from build123d import *

# Parameters (mm, degrees)
SKETCH_1_R      = 925
SKETCH_1_W      = 122
SKETCH_1_H      = 122
EXTRUDE_1_DEPTH = 12


with BuildPart() as part:
    # 草图1 → 凸台-拉伸1 (new body)
    with BuildSketch(Plane(origin=(0, 0, 0), x_dir=(1, 0, 0), z_dir=(0, 1, 0))):
        with Locations(Location((0, 0, 0), (0, 0, 270))):
            Circle(SKETCH_1_R)
        with BuildLine():
            Line((-648.074069841, 425), (-425, 425))
            Line((-425, 425), (-425, 648.074069841))
            ThreePointArc((-425, 648.074069841), (0, 775), (425, 648.074069841))
            Line((425, 648.074069841), (425, 425))
            Line((425, 425), (648.074069841, 425))
            ThreePointArc((648.074069841, 425), (775, 0), (648.074069841, -425))
            Line((648.074069841, -425), (425, -425))
            Line((425, -425), (425, -648.074069841))
            ThreePointArc((425, -648.074069841), (0, -775), (-425, -648.074069841))
            Line((-425, -648.074069841), (-425, -425))
            Line((-425, -425), (-648.074069841, -425))
            ThreePointArc((-648.074069841, -425), (-775, 0), (-648.074069841, 425))
        make_face(mode=Mode.SUBTRACT)
        with Locations((-550, 550)):
            Rectangle(SKETCH_1_W, SKETCH_1_H, mode=Mode.SUBTRACT)
        with Locations((-550, -550)):
            Rectangle(SKETCH_1_W, SKETCH_1_H, mode=Mode.SUBTRACT)
        with Locations((550, -550)):
            Rectangle(SKETCH_1_W, SKETCH_1_H, mode=Mode.SUBTRACT)
        with Locations((550, 550)):
            Rectangle(SKETCH_1_W, SKETCH_1_H, mode=Mode.SUBTRACT)
    extrude(amount=EXTRUDE_1_DEPTH)


solid = part.part
Read the model definition and answer for the solid it produces. Units are mm, in the model's axes. A direction names the side the tool comes from. Coordinates: 2 decimals unless noted, no trailing zeros. Order: outer loops, then holes, each group sorted by start corner. A loop starts at its lowest first (then second) coordinate and runs counter-clockwise, first axis right, second up. Notation, with made-up numbers: M 59,-21 L 92,-21 A15 ccw 92,5 Z; hole C -33,68.25 d9. An arc over 180 degrees is marked long. Put each result on its own line as item: value. Start each with the question number.
Item 1: Section B-B, the plane y = 6.5 is taken. Count the separate pieces of the cut face and the enclosed holes in it, plus the area to 3 significant figures.
Item 2: Given pin 1 Ø6 at (y, z) = (8.5, -547) entering from +X; pin 2 Ø5 at (x, y) = (-506, 5.5) entering from +Z; pin 3 Ø6 at (y, z) = (5, 545.5) entering from +X, each flat-ended and moving along its own axis, determine where each tip first touches the part or whether it passes through.
Item 3: Section A-A, the plane x = 0 is taken. Determine the outline of the cut face in (y, z).
Item 4: Consider probe 1 along Z at (x, y) = (-8, 3.75); probe 2 along Z at (x, y) = (-523.5, 9.5); probe 3 along X at (y, z) = (11.25, -12.5). Determine where each line is inside the solid, lowest interval first. Write a range as [from, to].
Item 5: For faces 4 (the face through (-475, 12, 475)), 5 (the face through (6.298, 5.916, 774.974)), determine the directions among +Z, -Z, +X, -X, +Y, -Y from which every point of the face is accessible in a straight line to the end or side of a thin tool.
Item 6: The mould has two halves that part along Z. Classify faces 1 (the face through (625.16, 5.92, -681.76)), 2 (the face through (-774.974, 5.916, 6.298)), 3 (the face through (-475, 0, 475)): +Z half, -Z half, draft (parallel to the pull), parting line (faces both ways), or undercut.
Item 7: Section C-C, the plane z = 0 is taken. Determine the outline of the cut face in (x, y).
Computed:
1. separate pieces: 1
1. enclosed holes: 5
1. area: 855,000 mm2
2. pin 1: stops at x = 748.12
2. pin 2: stops at z = 775.96
2. pin 3: stops at x = 749.21
3. outline: M 0,-925 L 12,-925 L 12,-775 L 0,-775 Z; M 0,775 L 12,775 L 12,925 L 0,925 Z
4. probe 1: z = [-924.97, -774.96], [774.96, 924.97]
4. probe 2: z = [-762.61, -611], [-489, -425], [425, 489], [611, 762.61]
4. probe 3: x = [-924.92, -774.9], [774.9, 924.92]
5. face 4: +Z, -Z, +X, -X, +Y
5. face 5: +Y, -Y
6. face 1: parting line
6. face 2: undercut
6. face 3: draft
7. outline: M -925,0 L -775,0 L -775,12 L -925,12 Z; M 775,0 L 925,0 L 925,12 L 775,12 Z
